```python
from build123d import *

# Parameters (mm, degrees)
SKETCH1_W                               = 345
SKETCH1_H                               = 220
BOSS_EXTRUDE1_DEPTH                     = 16
CBORE_FOR_M5_HEX_HEAD_BOLT1_D           = 5.5
CBORE_FOR_M5_HEX_HEAD_BOLT1_CBORE_D     = 10
CBORE_FOR_M5_HEX_HEAD_BOLT1_CBORE_DEPTH = 6
SKETCH4_W                               = 62.700686025
SKETCH4_H                               = 220
SKETCH4_W_2                             = 51.921757643
CUT_EXTRUDE1_DEPTH                      = 2
M8_TAPPED_HOLE1_D                       = 6.8


with BuildPart() as part:
    # Sketch1 → Boss-Extrude1 (new body)
    with BuildSketch(Plane(origin=(0, 0, 0), x_dir=(1, 0, 0), z_dir=(0, 1, 0))):
        Rectangle(SKETCH1_W, SKETCH1_H)
    extrude(amount=BOSS_EXTRUDE1_DEPTH)

    # CBORE for M5 Hex Head Bolt1 (through all)
    with Locations(Plane(origin=(0, 16, 0), x_dir=(1, 0, 0), z_dir=(0, 1, 0))):
        with Locations((160.5, 95.483075679), (128.5, 95.483075679), (128.5, 59.483075679), (160.5, 59.483075679), (160.5, -43.516924321), (160.5, -79.516924321), (128.5, -79.516924321), (-91.5, -51.5), (-59.5, -51.5), (-59.5, -87.5), (-91.5, -87.5), (-91.5, 59.483075679), (-59.5, 59.483075679), (-59.5, 95.483075679), (-91.5, 95.483075679)):
            CounterBoreHole(CBORE_FOR_M5_HEX_HEAD_BOLT1_D / 2, CBORE_FOR_M5_HEX_HEAD_BOLT1_CBORE_D / 2, CBORE_FOR_M5_HEX_HEAD_BOLT1_CBORE_DEPTH)

    # Sketch4 → Cut-Extrude1 (cut)
    with BuildSketch(Plane.XZ):
        with Locations((-73.793884323, 0)):
            Rectangle(SKETCH4_W, SKETCH4_H)
        with Locations((146.539121179, 0)):
            Rectangle(SKETCH4_W_2, SKETCH4_H)
    extrude(amount=-CUT_EXTRUDE1_DEPTH, mode=Mode.SUBTRACT)

    # M8 Tapped Hole1 (through all)
    with Locations(Plane(origin=(0, 0, 0), x_dir=(-1, 0, 0), z_dir=(0, -1, 0))):
        with Locations((-59.5, 25), (-9.5, 25), (-9.5, -25), (-59.5, -25)):
            Hole(M8_TAPPED_HOLE1_D / 2)


solid = part.part
```
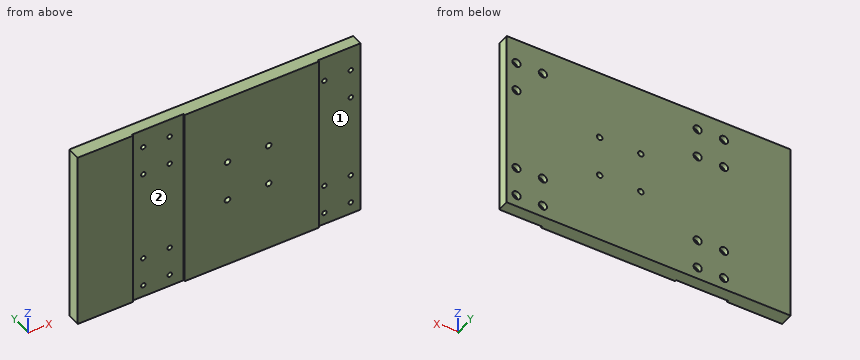
Can you work these out from the model? Positions are in its coordinate system, mm. Face numbers are marked on the shaded views. Coordinates: 2 decimals unless noted, no trailing zeros. Loops run counter-clockwise (first coordinate to the right, second up) from the corner with the lowest first, then second, coordinate; pieces in that order, holes last.
1) I need wall thicknesses on probe 1 along Z at (x, y) = (9.5, 6.75); probe 2 along Z at (x, y) = (-60, 8.25); probe 3 along Z at (x, y) = (160.5, 5.25). Which ranges of each line are inside material? Lowest first, please.
2) Thinking about a two-plate mould opening in X: for the marked faces 1 and 2, which applies, pulls with the +X half, pulls with the -X half, needs draft (parallel to the pull), parting line crosses it, or undercut?
3) For pin 1 (9 mm diameter, centred on x = 160.5, z = 79.52, fed in from +Y); pin 2 (11.5 mm diameter, centred on x = 160.5, z = -59.48, fed in from -Y); pin 3 (6 mm diameter, centred on x = 59.5, z = -25, fed in from -Y), each with a flat end and sliding along its axis, tell me the tip position at first contact or that it passes through.
4) Imagine slicing it at A-A on z = 25. List the corners of the cut face in (x, y) for me, plus the area to 3 significant figures.
5) Imagine slicing it at B-B on x = 9.5. List the corners of the cut face in (y, z) for me, plus the area to 3 significant figures.
Completed:
1. probe 1: z = -110 to -28.4, -21.6 to 21.6, 28.4 to 110
1. probe 2: z = -110 to -98.19, -92.78 to -62.19, -56.78 to 48.8, 54.2 to 84.8, 90.2 to 110
1. probe 3: z = -110 to -98.23, -92.73 to -62.23, -56.73 to 40.77, 46.27 to 76.77, 82.27 to 110
2. face 1: needs draft
2. face 2: undercut
3. pin 1: stops at y = 10
3. pin 2: stops at y = 2
3. pin 3: passes through
4. outline: (-172.5, 0) - (-105.14, 0) - (-105.14, 2) - (-42.44, 2) - (-42.44, 0) - (6.1, 0) - (6.1, 16) - (-172.5, 16) - close; (12.9, 0) - (56.1, 0) - (56.1, 16) - (12.9, 16) - close; (62.9, 0) - (120.58, 0) - (120.58, 2) - (172.5, 2) - (172.5, 16) - (62.9, 16) - close
4. area: 5,070 mm2
5. outline: (0, -110) - (16, -110) - (16, -28.4) - (0, -28.4) - close; (0, -21.6) - (16, -21.6) - (16, 21.6) - (0, 21.6) - close; (0, 28.4) - (16, 28.4) - (16, 110) - (0, 110) - close
5. area: 3,300 mm2
